```python
from build123d import *

# Parameters (mm, degrees)
SKETCH1_W                                            = 22
SKETCH1_H                                            = 10
BOSS_EXTRUDE1_DEPTH                                  = 8
CBORE_FOR_M4_HEXAGON_SOCKET_HEAD_CAP_SCR_D           = 4.5
CBORE_FOR_M4_HEXAGON_SOCKET_HEAD_CAP_SCR_CBORE_D     = 8
CBORE_FOR_M4_HEXAGON_SOCKET_HEAD_CAP_SCR_CBORE_DEPTH = 4.6
SKETCH4_W                                            = 8
SKETCH4_H                                            = 7
BOSS_EXTRUDE2_DEPTH                                  = 8
M4_TAPPED_HOLE1_D                                    = 3.3
FILLET1_R                                            = 2
CHAMFER1_SIZE                                        = 1


with BuildPart() as part:
    # Sketch1 → Boss-Extrude1 (new body)
    with BuildSketch(Plane.XY):
        Rectangle(SKETCH1_W, SKETCH1_H)
    extrude(amount=BOSS_EXTRUDE1_DEPTH)

    # CBORE for M4 Hexagon socket head cap screws1 (through all)
    with Locations(Plane(origin=(0, 0, 0), x_dir=(-1, 0, 0), z_dir=(0, 0, -1))):
        with Locations((-6.5, 0), (6.5, 0)):
            CounterBoreHole(CBORE_FOR_M4_HEXAGON_SOCKET_HEAD_CAP_SCR_D / 2, CBORE_FOR_M4_HEXAGON_SOCKET_HEAD_CAP_SCR_CBORE_D / 2, CBORE_FOR_M4_HEXAGON_SOCKET_HEAD_CAP_SCR_CBORE_DEPTH)

    # Sketch4 → Boss-Extrude2 (add)
    with BuildSketch(Plane(origin=(0, 0, 0), x_dir=(-1, 0, 0), z_dir=(0, 0, -1))):
        with Locations((0, 8.5)):
            Rectangle(SKETCH4_W, SKETCH4_H)
    extrude(amount=-BOSS_EXTRUDE2_DEPTH)

    # M4 Tapped Hole1 (through all)
    with Locations(Plane(origin=(0, 0, 0), x_dir=(-1, 0, 0), z_dir=(0, 0, -1))):
        with Locations((0, 8.5)):
            Hole(M4_TAPPED_HOLE1_D / 2)

    # Fillet1
    fillet1_edges = [part.edges().sort_by_distance(p)[0] for p in [
        (4, 5, 4),
        (-4, 5, 4),
    ]]
    fillet(fillet1_edges, radius=FILLET1_R)

    # Chamfer1
    chamfer1_edges = [part.edges().sort_by_distance(p)[0] for p in [
        (4, 12, 4),
        (-4, 12, 4),
        (11, -5, 4),
        (-11, -5, 4),
        (-11, 5, 4),
        (11, 5, 4),
    ]]
    chamfer(chamfer1_edges, length=CHAMFER1_SIZE)


solid = part.part
```
Model file for the job. Use its own axes, mm. A direction names the side the tool comes from. Coordinates: 2 decimals unless noted, no trailing zeros. Write each loop counter-clockwise with the first axis right and the second up, starting at its lowest first coordinate (ties: lowest second). Pieces come first, ordered by that corner, then holes. Notation, with made-up numbers: (45, 78) - (102, 78) arc R25 ccw to (102, 116) - close; hole circle Ø9 at (21.5, -3.75). An arc over 180 degrees is marked (long way). One line per item, written item: value. Start each with the question number.
1. Tool access for faces 1 (the flat face through (8, 5, 4)), 2 (the flat face through (0, 2, 0)), 3 (the flat face through (-8, 5, 4)): list every direction of +Z, -Z, +X, -X, +Y, -Y with a clear straight run to the whole face (end or side of a thin tool).
2. Slice it at D-D (x = -6.5). Write the cut outline in (y, z), plus the area to 3 significant figures.
3. Slice it at A-A (y = 8.5). Write the cut outline in (x, z).
4. Mould opens along Y. For faces 4 (the flat face through (-10.5, 4.5, 3.9)), 5 (the flat face through (-10.5, -4.5, 3.9)), 6 (the flat face through (5, -2, 4.6)), 7 (the flat face through (-4, 9, 4)) say: released by +Y, released by -Y, zero draft, split by the parting line, or undercut.
5. Slice it at B-B (z = 6.5). Write the cut outline in (x, y), plus the area to 3 significant figures.
6. Flat gauge pins, fed straight in: pin 1 (1.2 mm diameter, centred on y = 9.5, z = 4, fed in from -X); pin 2 (2 mm diameter, centred on x = 7.5, z = 3.5, fed in from +Y); pin 3 (2 mm diameter, centred on y = 10, z = 4, fed in from +X). Where does each tip first touch, or does it go through?
7. Slice it at C-C (y = 0). Write the cut outline in (x, z), plus the area to 3 significant figures.
8. Probe line 1 (Y direction, x = 6.5, z = 7); line 2 (Y direction, x = 0, z = 2.25); line 3 (X direction, y = 2, z = 5.25). List the from-to ranges inside material, lowest first. Write a range as from..to.
Answers below:
1. face 1: +Z, -Z, +X, +Y
1. face 2: -Z, +X, -X, +Y, -Y
1. face 3: +Z, -Z, -X, +Y
2. outline: (-5, 0) - (-4, 0) - (-4, 4.6) - (-2.25, 4.6) - (-2.25, 8) - (-5, 8) - close; (2.25, 4.6) - (4, 4.6) - (4, 0) - (5, 0) - (5, 8) - (2.25, 8) - close
2. area: 27.9 mm^2
3. outline: (-4, 0) - (-1.65, 0) - (-1.65, 8) - (-4, 8) - close; (1.65, 0) - (4, 0) - (4, 8) - (1.65, 8) - close
4. face 4: released by +Y
4. face 5: released by -Y
4. face 6: undercut
4. face 7: zero draft
5. outline: (-11, -4) - (-10, -5) - (10, -5) - (11, -4) - (11, 4) - (10, 5) - (6, 5) arc R2 cw to (4, 7) - (4, 11) - (3, 12) - (-3, 12) - (-4, 11) - (-4, 7) arc R2 cw to (-6, 5) - (-10, 5) - (-11, 4) - close; hole circle Ø4.5 at (-6.5, 0); hole circle Ø3.3 at (0, 8.5); hole circle Ø4.5 at (6.5, 0)
5. area: 234 mm^2
6. pin 1: stops at x = -4
6. pin 2: stops at y = 5
6. pin 3: stops at x = 4
7. outline: (-11, 0) - (-10.5, 0) - (-10.5, 4.6) - (-8.75, 4.6) - (-8.75, 8) - (-11, 8) - close; (-4.25, 4.6) - (-2.5, 4.6) - (-2.5, 0) - (2.5, 0) - (2.5, 4.6) - (4.25, 4.6) - (4.25, 8) - (-4.25, 8) - close; (8.75, 4.6) - (10.5, 4.6) - (10.5, 0) - (11, 0) - (11, 8) - (8.75, 8) - close
7. area: 71.8 mm^2
8. line 1: y = -5..-2.25, 2.25..5
8. line 2: y = -5..6.85, 10.15..12
8. line 3: x = -11..-7.53, -5.47..5.47, 7.53..11
